from build123d import *

# Parameters (mm, degrees)
BASE_PLATE_SKETCH_W             = 100
BASE_PLATE_SKETCH_H             = 20
BASE_PLATE_DEPTH                = 100
MOUNTING_FLANGE_SKETCH_W        = 100
MOUNTING_FLANGE_SKETCH_H        = 100
MOUNTING_FLANGE_DEPTH           = 10
FLANGE_CORNER_CHAMFER_20MM_SIZE = 20
LUG_PROFILE_SKETCH_R            = 10
UPRIGHT_LUG_DEPTH               = 10
ADJUSTMENT_SLOTS_2X_DEPTH       = 166
MOUNTING_HOLES_SKETCH_R         = 5
FLANGE_MOUNTING_HOLES_DEPTH     = 10


with BuildPart() as part:
    # Base Plate Sketch → Base Plate (new body)
    with BuildSketch(Plane.XY):
        with Locations((50, 10)):
            Rectangle(BASE_PLATE_SKETCH_W, BASE_PLATE_SKETCH_H)
    extrude(amount=BASE_PLATE_DEPTH)

    # Mounting Flange Sketch → Mounting Flange (add)
    with BuildSketch(Plane(origin=(0, 0, 0), x_dir=(1, 0, 0), z_dir=(0, 1, 0))):
        with Locations((-50, -50)):
            Rectangle(MOUNTING_FLANGE_SKETCH_W, MOUNTING_FLANGE_SKETCH_H)
    extrude(amount=MOUNTING_FLANGE_DEPTH)

    # Flange Corner Chamfer 20mm
    flange_corner_chamfer_20mm_edges = [part.edges().sort_by_distance(p)[0] for p in [
        (-100, 5, 0),
        (-100, 5, 100),
    ]]
    chamfer(flange_corner_chamfer_20mm_edges, length=FLANGE_CORNER_CHAMFER_20MM_SIZE)

    # Lug Profile Sketch → Upright Lug (add)
    with BuildSketch(Plane(origin=(100, 0, 0), x_dir=(0, 0, -1), z_dir=(1, 0, 0))):
        with BuildLine():
            Line((-100, 20), (-73.318010558, 89.015008798))
            ThreePointArc((-73.318010558, 89.015008798), (-50, 105), (-26.681989442, 89.015008798))
            Line((-26.681989442, 89.015008798), (0, 20))
            Line((0, 20), (-100, 20))
        make_face()
        with Locations((-50, 80)):
            Circle(LUG_PROFILE_SKETCH_R, mode=Mode.SUBTRACT)
    extrude(amount=-UPRIGHT_LUG_DEPTH)

    # Adjustment Slots Sketch → Adjustment Slots 2x (cut, through all)
    with BuildSketch(Plane(origin=(0, 20, 0), x_dir=(1, 0, 0), z_dir=(0, 1, 0))):
        with BuildLine():
            Line((10, -14), (60, -14))
            ThreePointArc((60, -14), (66, -20), (60, -26))
            Line((60, -26), (10, -26))
            ThreePointArc((10, -26), (4, -20), (10, -14))
        make_face()
        with BuildLine():
            Line((60, -86), (10, -86))
            ThreePointArc((10, -86), (4, -80), (10, -74))
            Line((10, -74), (60, -74))
            ThreePointArc((60, -74), (66, -80), (60, -86))
        make_face()
    extrude(amount=-ADJUSTMENT_SLOTS_2X_DEPTH, mode=Mode.SUBTRACT)

    # Mounting Holes Sketch → Flange Mounting Holes (cut)
    with BuildSketch(Plane(origin=(0, 10, 0), x_dir=(1, 0, 0), z_dir=(0, 1, 0))):
        with Locations(Location((-20, -25, 0), (0, 0, 270))):
            Circle(MOUNTING_HOLES_SKETCH_R)
        with Locations(Location((-60, -25, 0), (0, 0, 270))):
            Circle(MOUNTING_HOLES_SKETCH_R)
        with Locations(Location((-20, -75, 0), (0, 0, 270))):
            Circle(MOUNTING_HOLES_SKETCH_R)
        with Locations(Location((-60, -75, 0), (0, 0, 270))):
            Circle(MOUNTING_HOLES_SKETCH_R)
    extrude(amount=-FLANGE_MOUNTING_HOLES_DEPTH, mode=Mode.SUBTRACT)


solid = part.part
Input: part model. Units: mm. Frame: model coordinates. A direction names the side the tool comes from. Coordinates: 2 decimals unless noted, no trailing zeros. Loops run counter-clockwise (first coordinate to the right, second up) from the corner with the lowest first, then second, coordinate; pieces in that order, holes last. Notation, with made-up numbers: (-24.75, 19.5) -> (16.25, 19.5) arc R14 ccw to (16.25, 46.5) -> close; hole circle Ø3 at (47, 21). An arc over 180 degrees is marked (long way). Write item = value, one per line. Start each with the question number.
Item 1: Cut plane B-B, the plane y = 74.5. Return loops of the section in (x, z).
Item 2: Reachability of faces 4 (the face through (-100, 5, 50)), 5 (the face through (-51, 10, 49)), 6 (the face through (66, 10, 20)) from +Z, -Z, +X, -X, +Y, -Y: full face, straight path, thin tool, end or side. Return the list, or none.
Item 3: Cut plane A-A, the plane x = 26. Return loops of the section in (y, z).
Item 4: Mould query, pull axis X, two halves, no side actions, for faces 1 (the face through (35, 10, 86)), 2 (the face through (100, 42, 49)), 3 (the face through (0, 15, 49)). Classes: pulls with the +X half, pulls with the -X half, needs draft (parallel to the pull), parting line crosses it, or undercut.
Item 5: Cut plane C-C, the plane z = 57.5. Return loops of the section in (x, y).
Item 6: Cut plane D-D, the plane x = -60. Return loops of the section in (y, z), plus the area to 3 significant figures.
Item 7: Material intervals for line 1 (X direction, y = 6, z = 75); line 2 (Y direction, x = 95, z = 50); line 3 (Y direction, x = -32.5, z = 49), sorted ascending.
Item 8: First-contact query: P1, Ø12, axis at y = 41.5, z = 38, coming from the -X side; P2, Ø3, axis at x = -36, z = 76, coming from the +Y side; P3, Ø11, axis at y = 16, z = 67, coming from the -X side. Flat tips, straight axial feed; report the tip coordinate or a pass-through.
Ans:
q1.outline = (90, 21.07) -> (100, 21.07) -> (100, 41.65) -> (90, 41.65) -> close; (90, 58.35) -> (100, 58.35) -> (100, 78.93) -> (90, 78.93) -> close
q2.face_4 = +Z, -Z, -X, +Y, -Y
q2.face_5 = +Z, -Z, -X, +Y
q2.face_6 = +Y, -Y
q3.outline = (0, 0) -> (20, 0) -> (20, 14) -> (0, 14) -> close; (0, 26) -> (20, 26) -> (20, 74) -> (0, 74) -> close; (0, 86) -> (20, 86) -> (20, 100) -> (0, 100) -> close
q4.face_1 = undercut
q4.face_2 = pulls with the +X half
q4.face_3 = pulls with the -X half
q5.outline = (-100, 0) -> (100, 0) -> (100, 73.39) -> (90, 73.39) -> (90, 20) -> (0, 20) -> (0, 10) -> (-100, 10) -> close; (90, 86.61) -> (100, 86.61) -> (100, 103.85) -> (90, 103.85) -> close
q6.outline = (0, 0) -> (10, 0) -> (10, 20) -> (0, 20) -> close; (0, 30) -> (10, 30) -> (10, 70) -> (0, 70) -> close; (0, 80) -> (10, 80) -> (10, 100) -> (0, 100) -> close
q6.area = 800 mm²
q7.line_1 = -100 to -65, -55 to -25, -15 to 6.68, 63.32 to 100
q7.line_2 = 0 to 70, 90 to 105
q7.line_3 = 0 to 10
q8.P1 = 90
q8.P2 = 10
q8.P3 = 0
